Geometry: final body of the model. Coordinates: model frame, mm. A direction names the side the tool comes from. Give positions to 0.01 mm unless a question says otherwise; leave off trailing zeros. Write each loop counter-clockwise with the first axis right and the second up, starting at its lowest first coordinate (ties: lowest second). Pieces come first, ordered by that corner, then holes. Notation, with made-up numbers: M 50,-10 L 100,-10 A14 ccw 100,-1 Z; hole C -9.75,35 d8. An arc over 180 degrees is marked long. One line per question, with ' | ' between items.
from build123d import *

# Parameters (mm, degrees)
CUT_EXTRUDE1_DEPTH = 2


with BuildPart() as part:
    # Sketch1 → Base-Revolve (revolve)
    with BuildSketch(Plane.XY, mode=Mode.PRIVATE) as base_revolve_sk:
        Polygon((0, 0), (12, 0), (12, 2), (11, 3), (0.402, 3), (0, 2.598), align=None)
    revolve(base_revolve_sk.sketch.rotate(Axis((-0.277777778, 0, 0), (1, 0, 0)), 90), axis=Axis((-0.277777778, 0, 0), (1, 0, 0)))

    # Sketch2 → Cut-Extrude1 (cut)
    with BuildSketch(Plane.ZY):
        Polygon((-0.86, -1.489563695), (0.86, -1.489563695), (1.72, 0), (0.86, 1.489563695), (-0.86, 1.489563695), (-1.72, 0), align=None)
    extrude(amount=-CUT_EXTRUDE1_DEPTH, mode=Mode.SUBTRACT)

    # Sketch4 → Cut-Revolve2 (revolve, cut)
    with BuildSketch(Plane.XY, mode=Mode.PRIVATE) as cut_revolve2_sk:
        Polygon((2, 1.489563695), (2.86, 0), (2, 0), align=None)
    revolve(cut_revolve2_sk.sketch.rotate(Axis((-0.277777778, 0, 0), (1, 0, 0)), 90), axis=Axis((-0.277777778, 0, 0), (1, 0, 0)), mode=Mode.SUBTRACT)


solid = part.part
(1) Draft query along Y for faces 3 (the face through (0.99, 0.76, -1.28)), 4 (the face through (5.63, -0.9, 2.86)), 5 (the face through (0, 2, 0)). Return one class per face: released by +Y, released by -Y, zero draft, split by the parting line, or undercut.
Working result:
face 3: undercut | face 4: split by the parting line | face 5: zero draft
(2) Set-up query: faces 1 (the face through (1, -1.49, 0)), 2 (the face through (12, 0, 0)). Return all of +Z, -Z, +X, -X, +Y, -Y with unobstructed straight access to the full face (end or side cutting, diameter ignored); none if empty.
Working result:
face 1: -X | face 2: +Z, -Z, +X, +Y, -Y
(3) First-contact query: P1, Ø1.4, axis at x = 1, z = -0.5, coming from the -Y side; P2, Ø1.5, axis at x = 2.5, z = 2.5, coming from the +Y side. Flat tips, straight axial feed; report the tip coordinate or a pass-through.
Working result:
P1: stops at y = -3 | P2: stops at y = 2.44
(4) Material intervals for L1, parallel to Y at x = 0.5, z = 1.35; L2, parallel to Y at x = 0.5, z = -0.75; L3, parallel to Z at x = 6, y = -2.4, sorted ascending. Write a range as [from, to].
Working result:
L1: y = [-2.68, -0.64], [0.64, 2.68] | L2: y = [-2.9, -1.49], [1.49, 2.9] | L3: z = [-1.8, 1.8]
(5) Cut plane A-A, the plane x = 7.25. Return loops of the section in (y, z).
Working result:
outline: C 0,0 d6
